Geometry: final body of the model. Coordinates: model frame, mm. Coordinates: 2 decimals unless noted, no trailing zeros. Write each loop counter-clockwise with the first axis right and the second up, starting at its lowest first coordinate (ties: lowest second). Pieces come first, ordered by that corner, then holes.
from build123d import *

# Parameters (mm, degrees)
SKETCH1_W                  = 600
SKETCH1_H                  = 720
BOSS_EXTRUDE1_DEPTH        = 8
F_17_0_17_DIAMETER_HOLE1_D = 17


with BuildPart() as part:
    # Sketch1 → Boss-Extrude1 (new, symmetric)
    with BuildSketch(Plane(origin=(0, 0, 0), x_dir=(1, 0, 0), z_dir=(0, 1, 0))):
        Rectangle(SKETCH1_W, SKETCH1_H)
    extrude(amount=BOSS_EXTRUDE1_DEPTH, both=True)

    # Ø17.0 (17) Diameter Hole1 (through all)
    with Locations(Plane(origin=(0, 8, 0), x_dir=(1, 0, 0), z_dir=(0, 1, 0))):
        with Locations((-275, -335), (-165, -335), (-55, -335), (55, -335), (165, -335), (275, -335), (-275, -201), (-275, -67), (-275, 67), (-275, 201), (-275, 335), (275, 335), (165, 335), (55, 335), (-55, 335), (-165, 335), (275, 201), (275, 67), (275, -67), (275, -201)):
            Hole(F_17_0_17_DIAMETER_HOLE1_D / 2)


solid = part.part
Item 1: Section B-B, the plane z = 335. Output: boundary loops of the cut face in (x, y), plus the area to 3 significant figures.
Derived:
outline: (-300, -8) - (-283.5, -8) - (-283.5, 8) - (-300, 8) - close; (-266.5, -8) - (-173.5, -8) - (-173.5, 8) - (-266.5, 8) - close; (-156.5, -8) - (-63.5, -8) - (-63.5, 8) - (-156.5, 8) - close; (-46.5, -8) - (46.5, -8) - (46.5, 8) - (-46.5, 8) - close; (63.5, -8) - (156.5, -8) - (156.5, 8) - (63.5, 8) - close; (173.5, -8) - (266.5, -8) - (266.5, 8) - (173.5, 8) - close; (283.5, -8) - (300, -8) - (300, 8) - (283.5, 8) - close
area: 7,970 mm2
Item 2: Section C-C, the plane z = 67. Output: boundary loops of the cut face in (x, y), plus the area to 3 significant figures.
Derived:
outline: (-300, -8) - (-283.5, -8) - (-283.5, 8) - (-300, 8) - close; (-266.5, -8) - (266.5, -8) - (266.5, 8) - (-266.5, 8) - close; (283.5, -8) - (300, -8) - (300, 8) - (283.5, 8) - close
area: 9,060 mm2
Item 3: Pin query (flat end, axial travel): pin 1 (19.5 mm diameter, centred on x = -275, z = 67, fed in from -Y). Return the tip coordinate at first contact, or that it passes through.
Derived:
pin 1: stops at y = -8
Item 4: Pull-direction query (Z, two-part tool) for faces 1 (the flat face through (-4, 0, -360)), 2 (the flat face through (-4, -8, -5)), 3 (the cylindrical face through (-268.255, -0.112, -195.828)); classes: released by +Z, released by -Z, zero draft, split by the parting line, or undercut.
Derived:
face 1: released by -Z
face 2: zero draft
face 3: undercut
Item 5: Section D-D, the plane x = 275. Output: boundary loops of the cut face in (y, z), plus the area to 3 significant figures.
Derived:
outline: (-8, -360) - (8, -360) - (8, -343.5) - (-8, -343.5) - close; (-8, -326.5) - (8, -326.5) - (8, -209.5) - (-8, -209.5) - close; (-8, -192.5) - (8, -192.5) - (8, -75.5) - (-8, -75.5) - close; (-8, -58.5) - (8, -58.5) - (8, 58.5) - (-8, 58.5) - close; (-8, 75.5) - (8, 75.5) - (8, 192.5) - (-8, 192.5) - close; (-8, 209.5) - (8, 209.5) - (8, 326.5) - (-8, 326.5) - close; (-8, 343.5) - (8, 343.5) - (8, 360) - (-8, 360) - close
area: 9,890 mm2
Item 6: Material intervals for probe 1 along Z at (x, y) = (-55, 2.25); probe 2 along X at (y, z) = (-2.25, 67); probe 3 along Z at (x, y) = (53.5, -6.25), sorted ascending.
Derived:
probe 1: z = -360 to -343.5, -326.5 to 326.5, 343.5 to 360
probe 2: x = -300 to -283.5, -266.5 to 266.5, 283.5 to 300
probe 3: z = -360 to -343.37, -326.63 to 326.63, 343.37 to 360
Item 7: Section A-A, the plane x = 165. Output: boundary loops of the cut face in (y, z), plus the area to 3 significant figures.
Derived:
outline: (-8, -360) - (8, -360) - (8, -343.5) - (-8, -343.5) - close; (-8, -326.5) - (8, -326.5) - (8, 326.5) - (-8, 326.5) - close; (-8, 343.5) - (8, 343.5) - (8, 360) - (-8, 360) - close
area: 11,000 mm2
